from build123d import *

# Parameters (mm, degrees)
PLATE_PROFILE_R         = 12.5
PLATE_PROFILE_R_2       = 3
PLATE_PROFILE_R_3       = 7.5
SUPPORT_PLATE_7MM_DEPTH = 7


with BuildPart() as part:
    # Plate Profile → Support Plate 7mm (new body)
    with BuildSketch(Plane.XY):
        with BuildLine():
            Line((-38, -32), (38, -32))
            ThreePointArc((38, -32), (53.238850443, -23.580054133), (54.221001351, -6.197493021))
            Line((54.221001351, -6.197493021), (16.221001351, 72.802506979))
            ThreePointArc((16.221001351, 72.802506979), (0, 83), (-16.221001351, 72.802506979))
            Line((-16.221001351, 72.802506979), (-54.221001351, -6.197493021))
            ThreePointArc((-54.221001351, -6.197493021), (-53.238850443, -23.580054133), (-38, -32))
        make_face()
        Circle(PLATE_PROFILE_R, mode=Mode.SUBTRACT)
        with Locations((0, -17.5)):
            Circle(PLATE_PROFILE_R_2, mode=Mode.SUBTRACT)
        with Locations((-15.155444566, 8.75)):
            Circle(PLATE_PROFILE_R_2, mode=Mode.SUBTRACT)
        with Locations((15.155444566, 8.75)):
            Circle(PLATE_PROFILE_R_2, mode=Mode.SUBTRACT)
        with Locations((-38, -14)):
            Circle(PLATE_PROFILE_R_3, mode=Mode.SUBTRACT)
        with Locations(Location((38, -14, 0), (0, 0, 180))):
            Circle(PLATE_PROFILE_R_3, mode=Mode.SUBTRACT)
        with Locations((0, 65)):
            Circle(PLATE_PROFILE_R_3, mode=Mode.SUBTRACT)
    extrude(amount=SUPPORT_PLATE_7MM_DEPTH)


solid = part.part
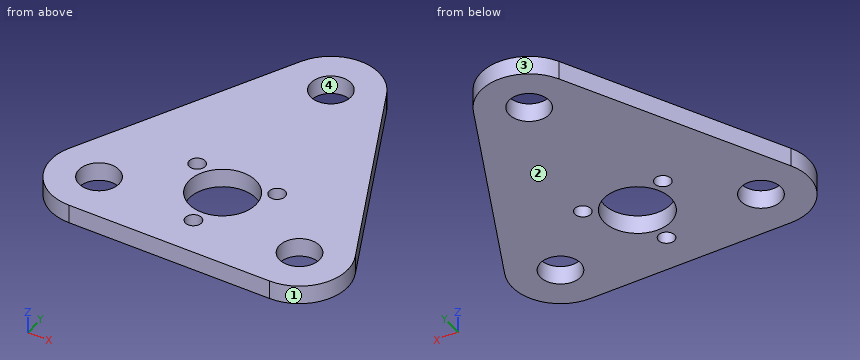
The listing builds one solid part. Answer for the finished solid, in the listing's coordinates (mm). Face numbers are marked on the shaded views. Round coordinates to 2 decimals unless told otherwise and drop trailing zeros. Write each loop counter-clockwise with the first axis right and the second up, starting at its lowest first coordinate (ties: lowest second). Pieces come first, ordered by that corner, then holes. Notation, with made-up numbers: M 19,64.25 L 78,64.25 A8 ccw 78,69.25 Z; hole C 1,26 d7. An arc over 180 degrees is marked long. Write each question's results on one line, items separated by ' | '. Start each with the question number.
Item 1: For a pull along X with two mould halves and no side action, classify the marked faces 1, 2, 3 and 4 as pulls with the +X half, pulls with the -X half, needs draft (parallel to the pull), parting line crosses it, or undercut.
Item 2: A cutting plane is placed at C-C on y = 61. Write down the section's boundary in (x, z).
Item 3: A cutting plane is placed at D-D on y = -17.5. Write down the section's boundary in (x, z).
Item 4: Straight lines are drawn through the part: L1, parallel to Y at x = 0, z = 2; L2, parallel to X at y = 6.5, z = 6.25; L3, parallel to X at y = 11.5, z = 1.75. For each, find the intervals that lie inside material, in ascending order. Write a range as [from, to].
Item 5: A cutting plane is placed at B-B on x = 0. Write down the section's boundary in (y, z), and give its area (3 significant figures).
Item 6: A cutting plane is placed at A-A on z = 2.75. Write down the section's boundary in (x, y).
Item 7: Flat-ended cylindrical pins translate along their axes: pin 1 Ø1 at (y, z) = (-6, 4) entering from +X; pin 2 Ø1.5 at (y, z) = (40, 3) entering from -X; pin 3 Ø1 at (y, z) = (-20.5, 3.5) entering from +X. Find the tip coordinate at first contact, or state that the pin passes through.
Check sheet entries:
1) face 1: pulls with the +X half | face 2: needs draft | face 3: parting line crosses it | face 4: undercut
2) outline: M -21.9,0 L -6.34,0 L -6.34,7 L -21.9,7 Z; M 6.34,0 L 21.9,0 L 21.9,7 L 6.34,7 Z
3) outline: M -55.66,0 L -44.63,0 L -44.63,7 L -55.66,7 Z; M -31.37,0 L -3,0 L -3,7 L -31.37,7 Z; M 3,0 L 31.37,0 L 31.37,7 L 3,7 Z; M 44.63,0 L 55.66,0 L 55.66,7 L 44.63,7 Z
4) L1: [-32, -20.5], [-14.5, -12.5], [12.5, 57.5], [72.5, 83] | L2: [-48.11, -17.14], [-13.17, -10.68], [10.68, 13.17], [17.14, 48.11] | L3: [-45.71, -16.35], [-13.96, -4.9], [4.9, 13.96], [16.35, 45.71]
5) outline: M -32,0 L -20.5,0 L -20.5,7 L -32,7 Z; M -14.5,0 L -12.5,0 L -12.5,7 L -14.5,7 Z; M 12.5,0 L 57.5,0 L 57.5,7 L 12.5,7 Z; M 72.5,0 L 83,0 L 83,7 L 72.5,7 Z | area: 483 mm²
6) outline: M -54.22,-6.2 A18 ccw -38,-32 L 38,-32 A18 ccw 54.22,-6.2 L 16.22,72.8 A18 ccw -16.22,72.8 Z; hole C -38,-14 d15; hole C -15.16,8.75 d6; hole C 0,0 d25; hole C 0,65 d15; hole C 0,-17.5 d6; hole C 15.16,8.75 d6; hole C 38,-14 d15
7) pin 1: x = 54.36 | pin 2: x = -32.36 | pin 3: x = 54.97
